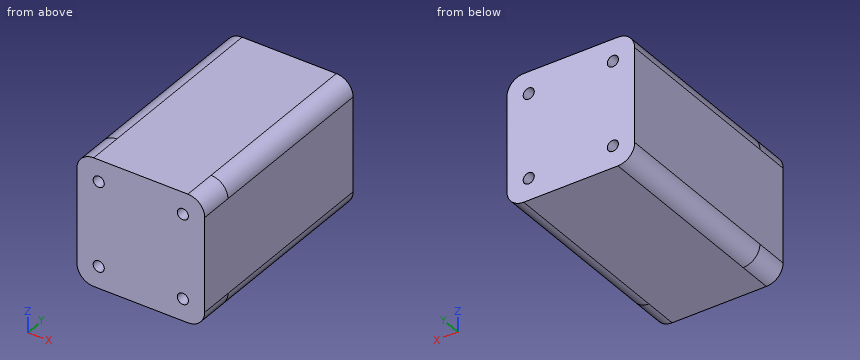
```python
from build123d import *

# Parameters (mm, degrees)
SKETCH1_W             = 38
SKETCH1_H             = 68
BOSS_EXTRUDE1_DEPTH   = 10
SKETCH2_W             = 38
SKETCH2_H             = 38
BOSS_EXTRUDE2_DEPTH   = 54
M4_TAPPED_HOLE2_D     = 3.3
M4_TAPPED_HOLE2_DEPTH = 10.1
M4_TAPPED_HOLE2_TIP   = 0.99142
FILLET1_R             = 5
M4_TAPPED_HOLE1_D     = 3.3
M4_TAPPED_HOLE1_DEPTH = 10.1
M4_TAPPED_HOLE1_TIP   = 0.99142
SKETCH8_OUTSIDE_W     = 60.164
SKETCH8_OUTSIDE_H     = 90.164
CUT_EXTRUDE1_DEPTH    = 75.919957


with BuildPart() as part:
    # Sketch1 → Boss-Extrude1 (new body)
    with BuildSketch(Plane(origin=(0, 0, 0), x_dir=(1, 0, 0), z_dir=(0, 1, 0))):
        Rectangle(SKETCH1_W, SKETCH1_H)
    extrude(amount=BOSS_EXTRUDE1_DEPTH)

    # Sketch2 → Boss-Extrude2 (add)
    with BuildSketch(Plane(origin=(0, 10, 0), x_dir=(1, 0, 0), z_dir=(0, 1, 0))):
        Rectangle(SKETCH2_W, SKETCH2_H)
    extrude(amount=BOSS_EXTRUDE2_DEPTH)

    # M4 Tapped Hole2
    with Locations(Plane.XZ):
        with Locations((-12.5, -12.5), (12.5, -12.5), (-12.5, 12.5), (12.5, 12.5)):
            Hole(M4_TAPPED_HOLE2_D / 2, depth=M4_TAPPED_HOLE2_DEPTH)
            with Locations((0, 0, -(M4_TAPPED_HOLE2_DEPTH + M4_TAPPED_HOLE2_TIP / 2))):  # 118° drill point
                Cone(0, M4_TAPPED_HOLE2_D / 2, M4_TAPPED_HOLE2_TIP, mode=Mode.SUBTRACT)

    # Fillet1
    fillet1_edges = [part.edges().sort_by_distance(p)[0] for p in [
        (19, 37, 19),
        (19, 37, -19),
        (-19, 37, -19),
        (-19, 37, 19),
        (19, 5, 34),
        (-19, 5, 34),
        (-19, 5, -34),
        (19, 5, -34),
    ]]
    fillet(fillet1_edges, radius=FILLET1_R)

    # M4 Tapped Hole1
    with Locations(Plane(origin=(0, 64, 0), x_dir=(1, 0, 0), z_dir=(0, 1, 0))):
        with Locations((-12.5, 12.5), (12.5, 12.5), (12.5, -12.5), (-12.5, -12.5)):
            Hole(M4_TAPPED_HOLE1_D / 2, depth=M4_TAPPED_HOLE1_DEPTH)
            with Locations((0, 0, -(M4_TAPPED_HOLE1_DEPTH + M4_TAPPED_HOLE1_TIP / 2))):  # 118° drill point
                Cone(0, M4_TAPPED_HOLE1_D / 2, M4_TAPPED_HOLE1_TIP, mode=Mode.SUBTRACT)

    # Sketch8 outside → Cut-Extrude1 (cut, through all)
    with BuildSketch(Plane(origin=(0, 64, 0), x_dir=(1, 0, 0), z_dir=(0, 1, 0))):
        Rectangle(SKETCH8_OUTSIDE_W, SKETCH8_OUTSIDE_H)
        with BuildLine():
            Line((-14, 19), (14, 19))
            ThreePointArc((14, 19), (17.535534, 17.535534), (19, 14))
            Line((19, 14), (19, -14))
            ThreePointArc((19, -14), (17.535534, -17.535534), (14, -19))
            Line((14, -19), (-14, -19))
            ThreePointArc((-14, -19), (-17.535534, -17.535534), (-19, -14))
            Line((-19, -14), (-19, 14))
            ThreePointArc((-19, 14), (-17.535534, 17.535534), (-14, 19))
        make_face(mode=Mode.SUBTRACT)
    extrude(amount=-CUT_EXTRUDE1_DEPTH, mode=Mode.SUBTRACT)


solid = part.part
```
Model file for the job. Use its own axes, mm. Round coordinates to 2 decimals unless told otherwise and drop trailing zeros. Write each loop counter-clockwise with the first axis right and the second up, starting at its lowest first coordinate (ties: lowest second). Pieces come first, ordered by that corner, then holes. Notation, with made-up numbers: (89.25, 26) - (123.25, 26) arc R31 cw to (123.25, 64) - close; hole circle Ø8 at (29, 60). An arc over 180 degrees is marked (long way). Use CSV: the item, a comma, the result in double quotes. Start each with the question number.
Item 1: Band-saw the part on A-A (z = 16.5). Write the cut outline in (x, y).
Item 2: Drill centre lines: L1, parallel to X at y = 59.75, z = -12.5; L2, parallel to Z at x = -14, y = 55. Where is each one in solid material? Low to high. Write a range as [from, to].
Item 3: Pin check, flat tips, straight feed: P1, Ø3, axis at x = 12.5, z = 12.5, coming from the -Y side; P2, Ø2, axis at x = 12.5, z = 12.5, coming from the -Y side. Stop position of each tip, or through.
Checked values:
1,outline,"(-18.33, 0) - (18.33, 0) - (18.33, 64) - (-18.33, 64) - close"
2,L1,"x = [-19, -14.15], [-10.85, 10.85], [14.15, 19]"
2,L2,"z = [-19, -13.19], [-11.81, 11.81], [13.19, 19]"
3,P1,"stops at y = 10.19"
3,P2,"stops at y = 10.49"
